```python
from build123d import *

# Parameters (mm, degrees)
BOSS_EXTRUDE1_DEPTH = 10


with BuildPart() as part:
    # Sketch1 → Boss-Extrude1 (new body)
    with BuildSketch(Plane.XY):
        Polygon((0, 0), (100, 0), (100, 60), (26, 360), (0, 360), align=None)
    extrude(amount=BOSS_EXTRUDE1_DEPTH)


solid = part.part
```
Could you check a few things on this model? Use its own coordinates, in mm. Coordinates: 2 decimals unless noted, no trailing zeros. Order: outer loops, then holes, each group sorted by start corner. A loop starts at its lowest first (then second) coordinate and runs counter-clockwise, first axis right, second up. Notation, with made-up numbers: M -24.5,4 L 6.5,4 A28 ccw 6.5,27 Z; hole C -31.5,43 d8. An arc over 180 degrees is marked long. Use one line per item in the form item = value. Start each with the question number.
1. Suppose I cut it at B-B on x = 46. Write out the boundary of the cut face in (y, z), then the cut area to 3 significant figures.
2. Please list where these lines run through material, in increasing order: line 1 (X direction, y = 224.5, z = 9.5); line 2 (X direction, y = 257, z = 3).
3. Suppose I cut it at C-C on y = 188. Write out the boundary of the cut face in (x, z).
4. Suppose I cut it at A-A on z = 2.25. Write out the boundary of the cut face in (x, y).
Geometry says:
q1.outline = M 0,0 L 278.92,0 L 278.92,10 L 0,10 Z
q1.area = 2,790 mm^2
q2.line_1 = 0 to 59.42
q2.line_2 = 0 to 51.41
q3.outline = M 0,0 L 68.43,0 L 68.43,10 L 0,10 Z
q4.outline = M 0,0 L 100,0 L 100,60 L 26,360 L 0,360 Z
